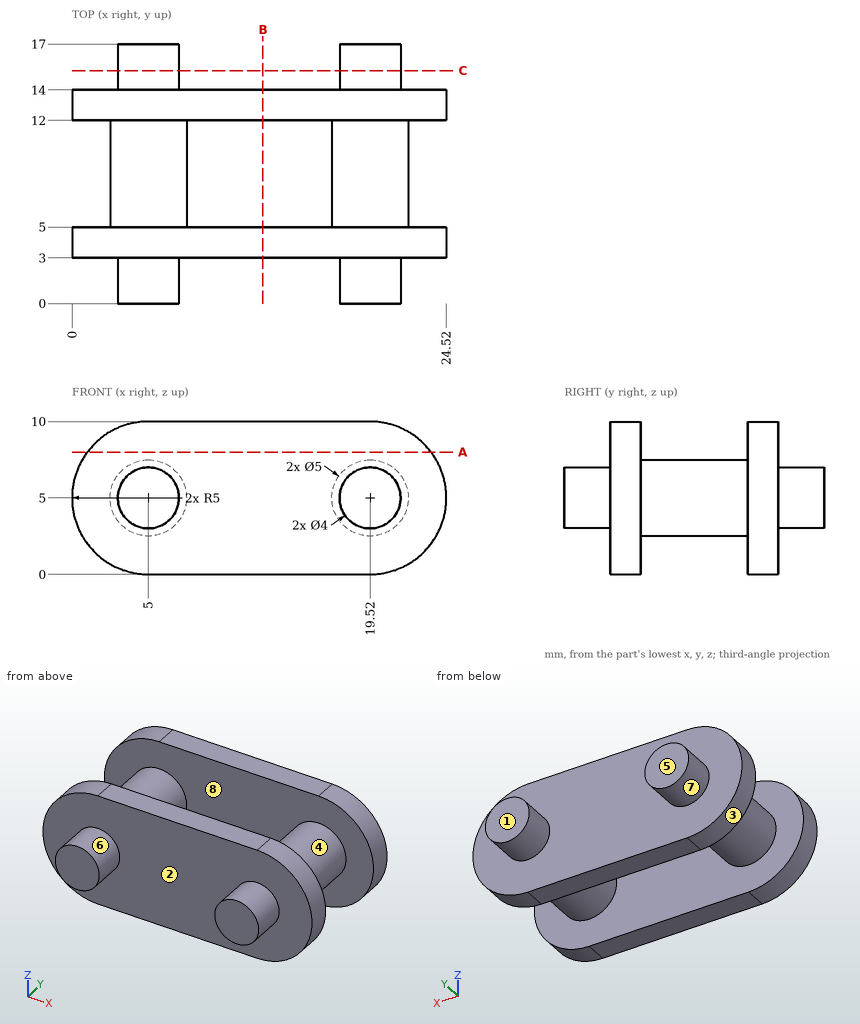
Can you work these out from the drawing? Everything is in mm from the part's minimum corner. A direction names the side the tool comes from. Coordinates: 2 decimals unless noted, no trailing zeros. Write each loop counter-clockwise with the first axis right and the second up, starting at its lowest first coordinate (ties: lowest second). Pieces come first, ordered by that corner, then holes. Notation, with made-up numbers: (42.25, 35) -> (46.25, 35) arc R32 ccw to (46.25, 66) -> close; hole circle Ø4 at (-7, 60.25). An arc over 180 degrees is marked (long way). Write each question's results on one line, items separated by ' | '. Start each with the question number.
Q1. Imagine slicing it at A-A (z = 8). Write out the boundary of the cut face in (x, y), then the cut area to 3 significant figures.
Q2. We'd pull the mould along Y, two halves only. Please class the marked faces 1, 2, 3 and 4: +Y half, -Y half, draft (parallel to the pull), parting line (faces both ways), or undercut.
Q3. I'm going to push flat-ended pins straight in: pin 1 (5 mm diameter, centred on x = 7.5, z = 7, fed in from -Y); pin 2 (4 mm diameter, centred on y = 8, z = 7.5, fed in from +X); pin 3 (4 mm diameter, centred on x = 21.5, y = 2, fed in from -Z); pin 4 (1.5 mm diameter, centred on x = 9, z = 6, fed in from -Y). Where does each tip first touch, or does it pass through?
Q4. On a 3-axis mill with a long thin cutter (end or side, diameter ignored), from which of +Z, -Z, +X, -X, +Y, -Y can I reach the whole of each face in a straight line? I mean the marked faces 5, 6, 7 and 8. Say none if no direction works.
Q5. Imagine slicing it at C-C (y = 15.25). Write out the boundary of the cut face in (x, z).
Q6. If I drill on probe 1 along X at (y, z) = (15, 5); probe 2 along Y at (x, z) = (11, 9.5); probe 3 along X at (y, z) = (6, 5.5), over which ranges is the centre line in solid material (lowest first)?
Q7. Imagine slicing it at B-B (x = 12.5). Write out the boundary of the cut face in (y, z).
Taken from the geometry:
1) outline: (1, 3) -> (23.52, 3) -> (23.52, 5) -> (1, 5) -> close; (1, 12) -> (23.52, 12) -> (23.52, 14) -> (1, 14) -> close | area: 90.1 mm^2
2) face 1: +Y half | face 2: -Y half | face 3: draft | face 4: undercut
3) pin 1: stops at y = 0 | pin 2: stops at x = 21.97 | pin 3: stops at z = 0.01 | pin 4: stops at y = 3
4) face 5: +Z, -Z, +X, -X, +Y | face 6: -Y | face 7: +Y | face 8: none
5) outline: circle Ø4 at (5, 5); circle Ø4 at (19.52, 5)
6) probe 1: x = 3 to 7, 17.52 to 21.52 | probe 2: y = 3 to 5, 12 to 14 | probe 3: x = 2.55 to 7.45, 17.07 to 21.97
7) outline: (3, 0) -> (5, 0) -> (5, 10) -> (3, 10) -> close; (12, 0) -> (14, 0) -> (14, 10) -> (12, 10) -> close
